Geometry: see drawing. Coordinates: mm, zero at the bounding-box minimum. Round coordinates to 2 decimals unless told otherwise and drop trailing zeros. Write each loop counter-clockwise with the first axis right and the second up, starting at its lowest first coordinate (ties: lowest second). Pieces come first, ordered by that corner, then holes. Notation, with made-up numbers: (75.25, 45) - (90.25, 45) arc R14 cw to (90.25, 63) - close; hole circle Ø3 at (13.5, 71.25). An arc over 180 degrees is marked (long way). One line per item, written item: value. Start each with the question number.
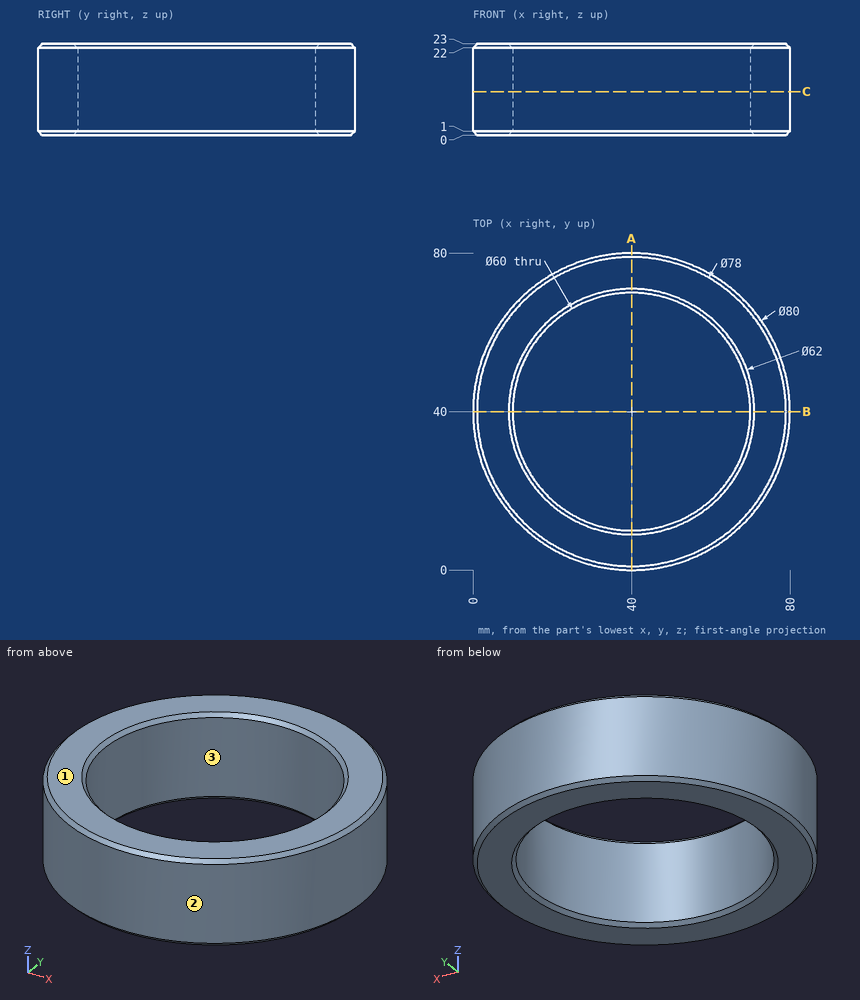
Q1. Cut plane C-C, the plane z = 11. Output: boundary loops of the cut face in (x, y).
Q2. Material intervals for probe 1 along X at (y, z) = (40.5, 1); probe 2 along X at (y, z) = (62, 9.25), sorted ascending. Write a range as from..to.
Q3. Cut plane A-A, the plane x = 40. Output: boundary loops of the cut face in (y, z), and give its area (3 significant figures).
Q4. Pull-direction query (Y, two-part tool) for the marked faces 1, 2 and 3; classes: pulls with the +Y half, pulls with the -Y half, needs draft (parallel to the pull), parting line crosses it, or undercut.
Q5. Contact query for flat-ended pins moving along their axis: pin 1 Ø2 at (y, z) = (14, 16.5) entering from +X (3 decimals); pin 2 Ø12 at (y, z) = (70, 18.5) entering from +X; pin 3 Ø1.5 at (x, z) = (13.5, 19) entering from +Y. Output: stop coordinate, or through.
A:
1. outline: circle Ø80 at (40, 40); hole circle Ø60 at (40, 40)
2. probe 1: x = 0..10, 70..80
2. probe 2: x = 6.59..19.6, 60.4..73.41
3. outline: (0, 1) - (1, 0) - (9, 0) - (10, 1) - (10, 22) - (9, 23) - (1, 23) - (0, 22) - close; (70, 1) - (71, 0) - (79, 0) - (80, 1) - (80, 22) - (79, 23) - (71, 23) - (70, 22) - close
3. area: 456 mm²
4. face 1: needs draft
4. face 2: parting line crosses it
4. face 3: undercut
5. pin 1: stops at x = 71.225
5. pin 2: stops at x = 72
5. pin 3: stops at y = 70.61
